```python
from build123d import *

# Parameters (mm, degrees)
SKETCH_1_W                  = 146
SKETCH_1_H                  = 636
EXTRUDE_1_DEPTH             = 1.5
SKETCH_2_W                  = 1.5
SKETCH_2_H                  = 636
EXTRUDE_2_DEPTH             = 109
SKETCH_4_W                  = 144.5
SKETCH_4_H                  = 1.5
EXTRUDE_4_DEPTH             = 66
EXTRUDE_5_DEPTH             = 730
SKETCH_6_W                  = 1.5
SKETCH_6_H                  = 634.5
EXTRUDE_6_DEPTH             = 20
SKETCH_7_W                  = 1.5
SKETCH_7_H                  = 730
EXTRUDE_7_DEPTH             = 10
SKETCH_8_W                  = 1.5
SKETCH_8_H                  = 56
EXTRUDE_8_DEPTH             = 10
SKETCH_10_W                 = 35
SKETCH_10_H                 = 150
CUT_EXTRUDE_2_DEPTH         = 2
HOLE_WIZARD_5_5_5_5_1_D     = 5.5
HOLE_WIZARD_5_5_5_5_2_D     = 5.5
HOLE_WIZARD_5_5_5_5_2_DEPTH = 1.5
HOLE_WIZARD_5_5_5_5_2_TIP   = 1.652366702
CUT_EXTRUDE_3_DEPTH         = 55


with BuildPart() as part:
    # 草图1 → 凸台-拉伸1 (new body)
    with BuildSketch(Plane.XY):
        with Locations((73, 318)):
            Rectangle(SKETCH_1_W, SKETCH_1_H)
    extrude(amount=EXTRUDE_1_DEPTH)

    # 草图2 → 凸台-拉伸2 (add)
    with BuildSketch(Plane.XY.offset(1.5)):
        with Locations((0.75, 318)):
            Rectangle(SKETCH_2_W, SKETCH_2_H)
    extrude(amount=EXTRUDE_2_DEPTH)

    # 草图4 → 凸台-拉伸4 (add)
    with BuildSketch(Plane.XY.offset(1.5)):
        with Locations((73.75, 0.75)):
            Rectangle(SKETCH_4_W, SKETCH_4_H)
    extrude(amount=EXTRUDE_4_DEPTH)

    # 草图5 → 凸台-拉伸5 (add)
    with BuildSketch(Plane.XZ):
        Polygon((0, 110.5), (0, 66), (146, 66), (146, 67.5), (1.5, 67.5), (1.5, 110.5), align=None)
    extrude(amount=EXTRUDE_5_DEPTH)

    # 草图6 → 凸台-拉伸6 (add)
    with BuildSketch(Plane(origin=(0, 0, 0), x_dir=(-1, 0, 0), z_dir=(0, 0, -1))):
        with Locations((-145.25, 318.75)):
            Rectangle(SKETCH_6_W, SKETCH_6_H)
    extrude(amount=EXTRUDE_6_DEPTH)

    # 草图7 → 凸台-拉伸7 (add)
    with BuildSketch(Plane(origin=(0, 0, 66), x_dir=(-1, 0, 0), z_dir=(0, 0, -1))):
        with Locations((-145.25, -365)):
            Rectangle(SKETCH_7_W, SKETCH_7_H)
    extrude(amount=EXTRUDE_7_DEPTH)

    # 草图8 → 凸台-拉伸8 (add)
    with BuildSketch(Plane.XZ):
        with Locations((145.25, 28)):
            Rectangle(SKETCH_8_W, SKETCH_8_H)
    extrude(amount=EXTRUDE_8_DEPTH)

    # 草图10 → 切除-拉伸2 (cut)
    with BuildSketch(Plane(origin=(1.5, 0, 0), x_dir=(0, 0, -1), z_dir=(1, 0, 0))):
        with Locations((-93, -655)):
            Rectangle(SKETCH_10_W, SKETCH_10_H)
    extrude(amount=-CUT_EXTRUDE_2_DEPTH, mode=Mode.SUBTRACT)

    # Ø5.5 (5.5) 直径孔1 (through all)
    with Locations(Plane(origin=(1.5, 0, 0), x_dir=(0, 0, -1), z_dir=(1, 0, 0))):
        with Locations((-86.5, 419), (-86.5, 169), (-86.5, -81), (-86.5, -331), (-86.5, -531)):
            Hole(HOLE_WIZARD_5_5_5_5_1_D / 2)

    # Ø5.5 (5.5) 直径孔2
    with Locations(Plane.ZY.offset(-144.5)):
        with Locations((-10, 301.5), (-10, 101.5)):
            Hole(HOLE_WIZARD_5_5_5_5_2_D / 2, depth=HOLE_WIZARD_5_5_5_5_2_DEPTH)
            with Locations((0, 0, -(HOLE_WIZARD_5_5_5_5_2_DEPTH + HOLE_WIZARD_5_5_5_5_2_TIP / 2))):  # 118° drill point
                Cone(0, HOLE_WIZARD_5_5_5_5_2_D / 2, HOLE_WIZARD_5_5_5_5_2_TIP, mode=Mode.SUBTRACT)

    # 草图15 → 切除-拉伸3 (cut)
    with BuildSketch(Plane.XY.offset(1.5)):
        Polygon((27, 636), (27, 630), (44, 630), (44, 501), (104, 501), (104, 630), (121, 630), (121, 636), align=None)
    extrude(amount=-CUT_EXTRUDE_3_DEPTH, mode=Mode.SUBTRACT)


solid = part.part
```
Geometry: final body of the model. Coordinates: model frame, mm. A direction names the side the tool comes from. Coordinates: 2 decimals unless noted, no trailing zeros. Order: outer loops, then holes, each group sorted by start corner. A loop starts at its lowest first (then second) coordinate and runs counter-clockwise, first axis right, second up. Notation, with made-up numbers: (41.25, 12.5) - (56.25, 12.5) arc R11 cw to (56.25, 17.5) - close; hole circle Ø5 at (7.25, 17). An arc over 180 degrees is marked (long way). Return JSON: item names as keys, results as strings. Group by question number.
1. Cut plane B-B (x = 88.5). Output: boundary loops of the cut face in (y, z), plus the area to 3 significant figures.
2. Pull-direction query (X, two-part tool) for faces 1 (the face through (146, 108, 1)), 2 (the face through (144.5, -363, 60)), 3 (the face through (71, 0, 33)); classes: pulls with the +X half, pulls with the -X half, needs draft (parallel to the pull), parting line crosses it, or undercut.
3. Pin query (flat end, axial travel): pin 1 (1 mm diameter, centred on y = -29.5, z = 86.5, fed in from +X); pin 2 (2 mm diameter, centred on x = 107.5, y = 388, fed in from +Z); pin 3 (1.2 mm diameter, centred on x = 34, z = 1, fed in from +Y); pin 4 (4.5 mm diameter, centred on y = 301.5, z = -10, fed in from -X). Return the tip coordinate at first contact, or that it passes through.
4. Set-up query: faces 4 (the face through (71, -360, 66)), 5 (the face through (75, -359, 67.5)), 6 (the face through (73, 1.5, 34)). Return all of +Z, -Z, +X, -X, +Y, -Y with unobstructed straight access to the full face (end or side cutting, diameter ignored); none if empty.
5. Cut plane A-A (y = -293). Output: boundary loops of the cut face in (x, z), plus the area to 4 significant figures.
6. Material intervals for line 1 along Y through (x, z) = (145, -10); line 2 along Y through (x, z) = (0.8, 86.5); line 3 along Z through (x, y) = (10, -334.5), sorted ascending. Write a range as [from, to].
Resolved:
{
 "1": {"outline": "(-730, 66) - (0, 66) - (0, 0) - (501, 0) - (501, 1.5) - (1.5, 1.5) - (1.5, 67.5) - (-730, 67.5) - close", "area": "1,950 mm²"},
 "2": {"face 1": "pulls with the +X half", "face 2": "pulls with the -X half", "face 3": "needs draft"},
 "3": {"pin 1": "stops at x = 1.5", "pin 2": "stops at z = 1.5", "pin 3": "stops at y = 630", "pin 4": "passes through"},
 "4": {"face 4": "-Z, -X, -Y", "face 5": "+Z, +X, +Y, -Y", "face 6": "+Z, +X, +Y"},
 "5": {"outline": "(0, 66) - (144.5, 66) - (144.5, 56) - (146, 56) - (146, 67.5) - (1.5, 67.5) - (1.5, 110.5) - (0, 110.5) - close", "area": "298.5 mm²"},
 "6": {"line 1": "y = [1.5, 98.75], [104.25, 298.75], [304.25, 636]", "line 2": "y = [-580, -533.75], [-528.25, -333.75], [-328.25, -83.75], [-78.25, 166.25], [171.75, 416.25], [421.75, 636]", "line 3": "z = [66, 67.5]"}
}
